Geometry: final body of the model. Coordinates: model frame, mm. A direction names the side the tool comes from. Round coordinates to 2 decimals unless told otherwise and drop trailing zeros. Loops run counter-clockwise (first coordinate to the right, second up) from the corner with the lowest first, then second, coordinate; pieces in that order, holes last. Notation, with made-up numbers: M 86,78 L 90,78 A25 ccw 90,107 Z; hole C 60,-8 d8. An arc over 180 degrees is marked long. Write each question's results on one line, items separated by ' | '.
```python
from build123d import *

# Parameters (mm, degrees)
SKETCH1_W           = 60
SKETCH1_H           = 60
SKETCH1_W_2         = 52
SKETCH1_H_2         = 52
BOSS_EXTRUDE1_DEPTH = 600
FILLET1_R           = 6
FILLET2_R           = 3


with BuildPart() as part:
    # Sketch1 → Boss-Extrude1 (new body)
    with BuildSketch(Plane.XY):
        Rectangle(SKETCH1_W, SKETCH1_H)
        Rectangle(SKETCH1_W_2, SKETCH1_H_2, mode=Mode.SUBTRACT)
    extrude(amount=BOSS_EXTRUDE1_DEPTH)

    # Fillet1
    fillet1_edges = [part.edges().sort_by_distance(p)[0] for p in [
        (30, -30, 300),
        (-30, -30, 300),
        (-30, 30, 300),
        (30, 30, 300),
    ]]
    fillet(fillet1_edges, radius=FILLET1_R)

    # Fillet2
    fillet2_edges = [part.edges().sort_by_distance(p)[0] for p in [
        (26, -26, 300),
        (26, 26, 300),
        (-26, 26, 300),
        (-26, -26, 300),
    ]]
    fillet(fillet2_edges, radius=FILLET2_R)


solid = part.part
```
1. Ray query, probe 1 along X at (y, z) = (-20.5, 190); probe 2 along Y at (x, z) = (24, 314). Return the intervals inside material, ascending.
Answer key:
probe 1: x = -30 to -26, 26 to 30 | probe 2: y = -30 to -25.83, 25.83 to 30
2. Draft query along Y for faces 1 (the face through (26, 0, 296)), 2 (the face through (0, -30, 296)), 3 (the face through (-27, 0, 600)). Return one class per face: pulls with the +Y half, pulls with the -Y half, needs draft (parallel to the pull), parting line crosses it, or undercut.
Answer key:
face 1: undercut | face 2: pulls with the -Y half | face 3: needs draft
3. Section B-B (x = -7.5). Output: boundary loops of the cut face in (y, z), then the cut area to 3 significant figures.
Answer key:
outline: M -30,0 L -26,0 L -26,600 L -30,600 Z; M 26,0 L 30,0 L 30,600 L 26,600 Z | area: 4,800 mm²
4. Section A-A (z = 509). Output: boundary loops of the cut face in (x, y), then the cut area to 3 significant figures.
Answer key:
outline: M -30,-24 A6 ccw -24,-30 L 24,-30 A6 ccw 30,-24 L 30,24 A6 ccw 24,30 L -24,30 A6 ccw -30,24 Z; hole M -26,-23 A3 ccw -23,-26 L 23,-26 A3 ccw 26,-23 L 26,23 A3 ccw 23,26 L -23,26 A3 ccw -26,23 Z | area: 873 mm²
5. Access query for faces 4 (the face through (30, 0, 296)), 5 (the face through (0, -26, 296)). Directions: +Z, -Z, +X, -X, +Y, -Y. A direction counts if a zero-diameter tool reaches every point of the face in a straight line with its end or side. Return the directions, or none.
Answer key:
face 4: +Z, -Z, +X, +Y, -Y | face 5: +Z, -Z
